Design review of the part built by this model. Coordinates are the model's own, in mm. A direction names the side the tool comes from. Coordinates: 2 decimals unless noted, no trailing zeros. Order: outer loops, then holes, each group sorted by start corner. A loop starts at its lowest first (then second) coordinate and runs counter-clockwise, first axis right, second up. Notation, with made-up numbers: (-33.5, 40) -> (-1.5, 40) arc R23 cw to (-1.5, 67) -> close; hole circle Ø1 at (26, -34.5). An arc over 180 degrees is marked (long way). Write item = value, one per line.
```python
from build123d import *

# Parameters (mm, degrees)
SKETCH_1_W             = 70
SKETCH_1_H             = 90
EXTRUDE_1_DEPTH        = 12
CUT_EXTRUDE_1_DEPTH    = 115.647285184
SKETCH_4_R             = 3.25
CUT_EXTRUDE_2_DEPTH    = 115.647285184
HOLE_WIZARD_M6_1_D     = 5
HOLE_WIZARD_M6_1_DEPTH = 17
HOLE_WIZARD_M6_1_TIP   = 1.502151548
SKETCH_11_R            = 2.75
CUT_EXTRUDE_3_DEPTH    = 115.647285255


with BuildPart() as part:
    # 草图1 → 凸台-拉伸1 (new body)
    with BuildSketch(Plane.XY):
        with Locations((35, -45)):
            Rectangle(SKETCH_1_W, SKETCH_1_H)
    extrude(amount=EXTRUDE_1_DEPTH)

    # 草图2 → 切除-拉伸1 (cut, through all)
    with BuildSketch(Plane.XY.offset(12)):
        with BuildLine():
            Line((20, -33), (50, -33))
            ThreePointArc((50, -33), (57, -40), (50, -47))
            Line((50, -47), (20, -47))
            ThreePointArc((20, -47), (13, -40), (20, -33))
        make_face()
    extrude(amount=-CUT_EXTRUDE_1_DEPTH, mode=Mode.SUBTRACT)

    # 草图4 → 切除-拉伸2 (cut, through all)
    with BuildSketch(Plane(origin=(70, 0, 0), x_dir=(0, 0, -1), z_dir=(1, 0, 0))):
        with Locations((-6, -40)):
            Circle(SKETCH_4_R)
    extrude(amount=-CUT_EXTRUDE_2_DEPTH, mode=Mode.SUBTRACT)

    # M6 螺纹孔1
    with Locations(Plane(origin=(0, 0, 0), x_dir=(1, 0, 0), z_dir=(0, 1, 0))):
        with Locations((62.5, -6), (7.5, -6)):
            Hole(HOLE_WIZARD_M6_1_D / 2, depth=HOLE_WIZARD_M6_1_DEPTH)
            with Locations((0, 0, -(HOLE_WIZARD_M6_1_DEPTH + HOLE_WIZARD_M6_1_TIP / 2))):  # 118° drill point
                Cone(0, HOLE_WIZARD_M6_1_D / 2, HOLE_WIZARD_M6_1_TIP, mode=Mode.SUBTRACT)

    # 草图11 → 切除-拉伸3 (cut, through all)
    with BuildSketch(Plane.XY.offset(12)):
        with Locations((10, -85)):
            Circle(SKETCH_11_R)
        with Locations((60, -85)):
            Circle(SKETCH_11_R)
    extrude(amount=-CUT_EXTRUDE_3_DEPTH, mode=Mode.SUBTRACT)


solid = part.part
```
(1) For faces 1 (the flat face through (70, -46, 6)), 2 (the cylindrical face through (60.19, -8.62, 6.96)), 3 (the flat face through (35, -47, 6)), list the 3-axis set-ups (+Z, -Z, +X, -X, +Y, -Y) from which the entire face can be reached by the end or side of a thin tool; tool diameter is ignored.
Report:
face_1 = +Z, -Z, +X, +Y, -Y
face_2 = +Y
face_3 = +Z, -Z
(2) The part is to be moulded in two halves that separate along Y. For faces 4 (the flat face through (35, -90, 6)), 5 (the cylindrical face through (56.524, -37.462, 8.751)), 6 (the flat face through (35, 0, 6)), say which applies: released by +Y, released by -Y, zero draft, split by the parting line, or undercut.
Report:
face_4 = released by -Y
face_5 = undercut
face_6 = released by +Y
(3) We need section D-D (y = -85). Write out the cut boundary in (x, z), and give its area (3 significant figures).
Report:
outline = (0, 0) -> (7.25, 0) -> (7.25, 12) -> (0, 12) -> close; (12.75, 0) -> (57.25, 0) -> (57.25, 12) -> (12.75, 12) -> close; (62.75, 0) -> (70, 0) -> (70, 12) -> (62.75, 12) -> close
area = 708 mm²
(4) We need section B-B (y = -40). Write out the cut boundary in (x, z).
Report:
outline = (0, 0) -> (13, 0) -> (13, 2.75) -> (0, 2.75) -> close; (0, 9.25) -> (13, 9.25) -> (13, 12) -> (0, 12) -> close; (57, 0) -> (70, 0) -> (70, 2.75) -> (57, 2.75) -> close; (57, 9.25) -> (70, 9.25) -> (70, 12) -> (57, 12) -> close
(5) We need section A-A (x = 21). Write out the cut boundary in (y, z), and give its area (3 significant figures).
Report:
outline = (-90, 0) -> (-47, 0) -> (-47, 12) -> (-90, 12) -> close; (-33, 0) -> (0, 0) -> (0, 12) -> (-33, 12) -> close
area = 912 mm²
(6) We need section C-C (z = 1). Write out the cut boundary in (x, y).
Report:
outline = (0, -90) -> (70, -90) -> (70, 0) -> (0, 0) -> close; hole circle Ø5.5 at (10, -85); hole (20, -47) -> (50, -47) arc R7 ccw to (50, -33) -> (20, -33) arc R7 ccw to start; hole circle Ø5.5 at (60, -85)
(7) For L1, parallel to Z at x = 61, y = -40; L2, parallel to Y at x = 30.5, z = 6.5; L3, parallel to Z at x = 62.5, y = -10.75, list the stretches that pass through material, from the lowest coordinate up.
Report:
L1 = 0 to 2.75, 9.25 to 12
L2 = -90 to -47, -33 to 0
L3 = 0 to 3.5, 8.5 to 12
(8) Insertion check: pin 1 (4.5 mm diameter, centred on x = 62.5, z = 6, fed in from +Y). The pin has a flat end and moves straight along its axis. Give the tip position at first contact, or say it passes through.
Report:
pin_1 = -17.15
